Print and shaded views of the part. All mm, measured from the part's lowest x, y and z. A direction names the side the tool comes from. Give positions to 0.01 mm unless a question says otherwise; leave off trailing zeros. Order: outer loops, then holes, each group sorted by start corner. A loop starts at its lowest first (then second) coordinate and runs counter-clockwise, first axis right, second up. Notation, with made-up numbers: (-35.5, -24) - (-18.5, -24) arc R19 cw to (-18.5, -5) - close; hole circle Ø9 at (-10, 43.5). An arc over 180 degrees is marked (long way). Answer in a Markdown table with one row per item.
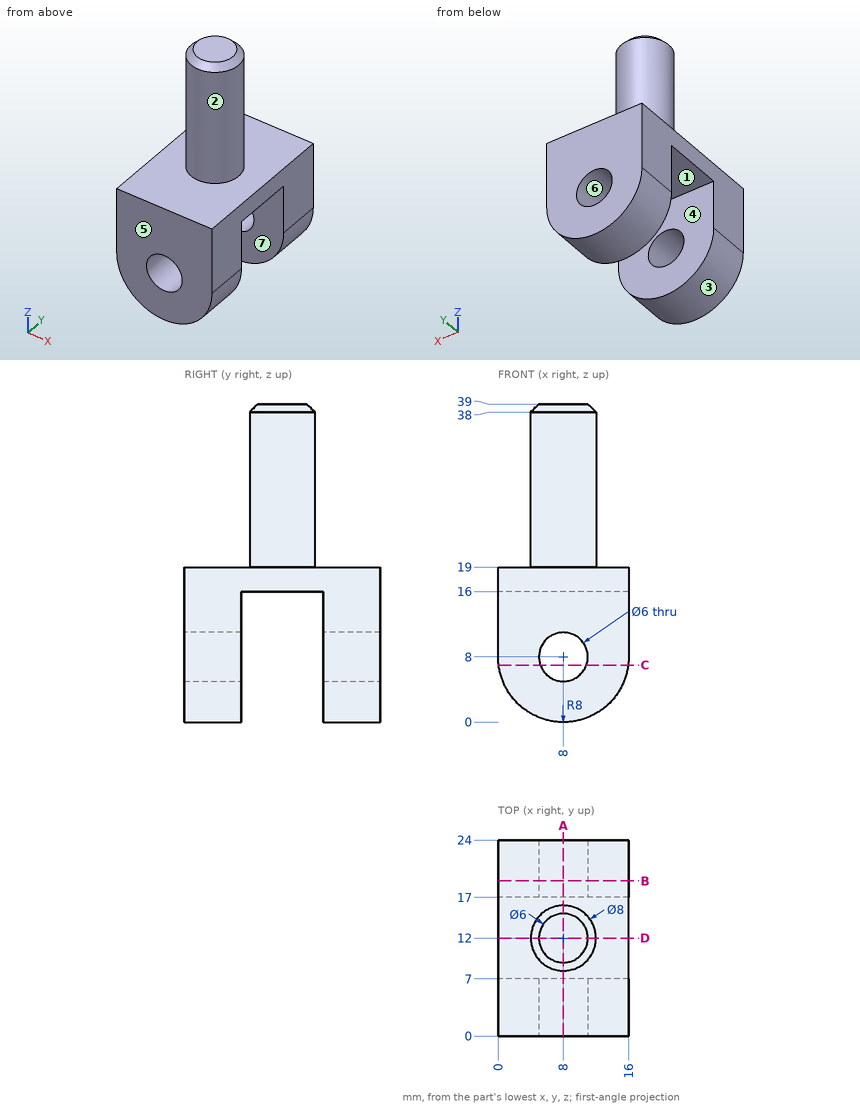
1. Cut at D-D on y = 12. Write the cut outline in (x, z).
Check result:
| item | result |
|---|---|
| outline | (0, 16) - (16, 16) - (16, 19) - (12, 19) - (12, 38) - (11, 39) - (5, 39) - (4, 38) - (4, 19) - (0, 19) - close |
2. Cut at C-C on z = 7. Write the cut outline in (x, y), and give its area (3 significant figures).
Check result:
| item | result |
|---|---|
| outline | (0.06, 0) - (5.17, 0) - (5.17, 7) - (0.06, 7) - close; (0.06, 17) - (5.17, 17) - (5.17, 24) - (0.06, 24) - close; (10.83, 0) - (15.94, 0) - (15.94, 7) - (10.83, 7) - close; (10.83, 17) - (15.94, 17) - (15.94, 24) - (10.83, 24) - close |
| area | 143 mm² |
3. Two-plate mould, pull along Y, no slides. Class the marked faces 4, 5, 6 and 7: +Y half, -Y half, draft (parallel to the pull), parting line (faces both ways), or undercut.
Check result:
| item | result |
|---|---|
| face 4 | undercut |
| face 5 | -Y half |
| face 6 | draft |
| face 7 | undercut |
4. Cut at B-B on y = 19. Write the cut outline in (x, z), and give its area (3 significant figures).
Check result:
| item | result |
|---|---|
| outline | (0, 8) arc R8 ccw to (16, 8) - (16, 19) - (0, 19) - close; hole circle Ø6 at (8, 8) |
| area | 248 mm² |
5. Cut at A-A on x = 8. Write the cut outline in (y, z), and give its area (3 significant figures).
Check result:
| item | result |
|---|---|
| outline | (0, 0) - (7, 0) - (7, 5) - (0, 5) - close; (0, 11) - (7, 11) - (7, 16) - (17, 16) - (17, 11) - (24, 11) - (24, 19) - (16, 19) - (16, 38) - (15, 39) - (9, 39) - (8, 38) - (8, 19) - (0, 19) - close; (17, 0) - (24, 0) - (24, 5) - (17, 5) - close |
| area | 371 mm² |
6. Probe line 1 (X direction, y = 20.25, z = 8); line 2 (Y direction, x = 10.75, z = 12); line 3 (Z direction, x = 13.5, y = 12.5). List the from-to ranges inside material, lowest first.
Check result:
| item | result |
|---|---|
| line 1 | x = 0 to 5, 11 to 16 |
| line 2 | y = 0 to 7, 17 to 24 |
| line 3 | z = 16 to 19 |
7. Which spindle directions (+Z, -Z, +X, -X, +Y, -Y) get a long thin tool onto all of the face, cutting with end or side? Do the marked faces 1, 2 and 3. Say none if no direction does.
Check result:
| item | result |
|---|---|
| face 1 | -Z, +X, -X |
| face 2 | +Z |
| face 3 | -Z, +Y, -Y |
8. Drop flat-ended pins along their axis: P1, Ø1, axis at x = 9, z = 34.5, coming from the +Y side; P2, Ø5, axis at x = 5, z = 10, coming from the -Y side; P3, Ø1, axis at x = 5.5, z = 34, coming from the +Y side; P4, Ø1.5, axis at x = 12.5, y = 2.5, coming from the -Z side. Give the stop position or say it passes through.
Check result:
| item | result |
|---|---|
| P1 | stops at y = 15.97 |
| P2 | stops at y = 0 |
| P3 | stops at y = 15.46 |
| P4 | stops at z = 0.93 |
